Geometry: final body of the model. Coordinates: model frame, mm. Face numbers are marked on the shaded views. A direction names the side the tool comes from. Give positions to 0.01 mm unless a question says otherwise; leave off trailing zeros. Write each loop counter-clockwise with the first axis right and the second up, starting at its lowest first coordinate (ties: lowest second). Pieces come first, ordered by that corner, then holes. Notation, with made-up numbers: (66, 74) - (80, 74) arc R9 ccw to (80, 89) - close; hole circle Ø9 at (60.25, 22.5). An arc over 180 degrees is marked (long way). Return JSON: item names as keys, results as strings.
from build123d import *

# Parameters (mm, degrees)
SKETCH_1_W                = 90
SKETCH_1_H                = 40
EXTRUDE_1_DEPTH           = 51
HOLE_WIZARD_1_D           = 11
HOLE_WIZARD_1_CBORE_D     = 18
HOLE_WIZARD_1_CBORE_DEPTH = 40
HOLE_WIZARD_M10_1_D       = 8.5
HOLE_WIZARD_M10_1_DEPTH   = 24.5
HOLE_WIZARD_M10_1_TIP     = 2.553657631


with BuildPart() as part:
    # 草图1 → 凸台-拉伸1 (new body)
    with BuildSketch(Plane(origin=(0, 0, 0), x_dir=(0, 0, -1), z_dir=(1, 0, 0))):
        Rectangle(SKETCH_1_W, SKETCH_1_H)
    extrude(amount=EXTRUDE_1_DEPTH)

    # 打孔尺寸(%根据)内六角圆柱头螺钉的类型1 (through all)
    with Locations(Plane(origin=(51, 0, 0), x_dir=(0, 0, -1), z_dir=(1, 0, 0))):
        with Locations((-20, 10), (20, 10), (-20, -10), (20, -10)):
            CounterBoreHole(HOLE_WIZARD_1_D / 2, HOLE_WIZARD_1_CBORE_D / 2, HOLE_WIZARD_1_CBORE_DEPTH)

    # M10 螺纹孔1
    with Locations(Plane(origin=(51, 0, 0), x_dir=(0, 0, -1), z_dir=(1, 0, 0))):
        with Locations((-35, 0), (35, 0)):
            Hole(HOLE_WIZARD_M10_1_D / 2, depth=HOLE_WIZARD_M10_1_DEPTH)
            with Locations((0, 0, -(HOLE_WIZARD_M10_1_DEPTH + HOLE_WIZARD_M10_1_TIP / 2))):  # 118° drill point
                Cone(0, HOLE_WIZARD_M10_1_D / 2, HOLE_WIZARD_M10_1_TIP, mode=Mode.SUBTRACT)


solid = part.part
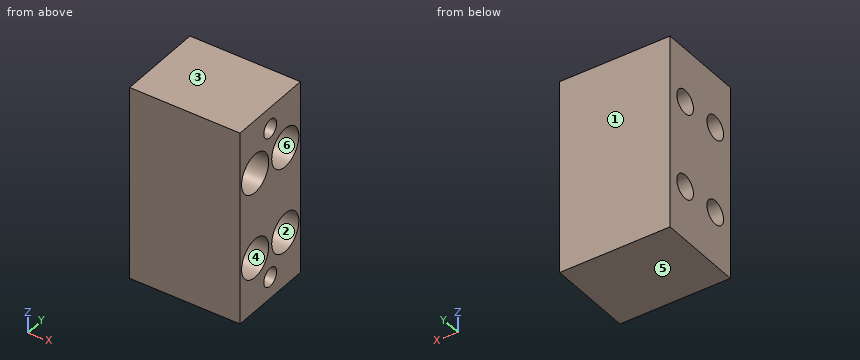
Q1. Section query D-D, the plane x = 8. Return the cut outline in (y, z), plus the area to 3 significant figures.
Answer key:
{"outline": "(-20, -45) - (20, -45) - (20, 45) - (-20, 45) - close; hole circle Ø11 at (-10, -20); hole circle Ø11 at (-10, 20); hole circle Ø11 at (10, -20); hole circle Ø11 at (10, 20)", "area": "3,220 mm^2"}
Q2. Pin query (flat end, axial travel): P1, Ø20.5, axis at y = 10, z = 20, coming from the +X side; P2, Ø5.5, axis at y = 7.5, z = 22.5, coming from the +X side; P3, Ø5, axis at y = 0, z = 35, coming from the +X side; P4, Ø10, axis at y = 10, z = 20, coming from the -X side. Return the tip coordinate at first contact, or that it passes through.
Answer key:
{"P1": "stops at x = 51", "P2": "stops at x = 11", "P3": "stops at x = 25.45", "P4": "passes through"}
Q3. Section query A-A, the plane y = 10. Return the cut outline in (x, z).
Answer key:
{"outline": "(0, -45) - (51, -45) - (51, -29) - (11, -29) - (11, -25.5) - (0, -25.5) - close; (0, -14.5) - (11, -14.5) - (11, -11) - (51, -11) - (51, 11) - (11, 11) - (11, 14.5) - (0, 14.5) - close; (0, 25.5) - (11, 25.5) - (11, 29) - (51, 29) - (51, 45) - (0, 45) - close"}
Q4. Section query B-B, the plane z = -20. Return the cut outline in (x, y), plus the area to 3 significant figures.
Answer key:
{"outline": "(0, -20) - (51, -20) - (51, -19) - (11, -19) - (11, -15.5) - (0, -15.5) - close; (0, -4.5) - (11, -4.5) - (11, -1) - (51, -1) - (51, 1) - (11, 1) - (11, 4.5) - (0, 4.5) - close; (0, 15.5) - (11, 15.5) - (11, 19) - (51, 19) - (51, 20) - (0, 20) - close", "area": "358 mm^2"}
Q5. Set-up query: the marked faces 5 and 6. Return all of +Z, -Z, +X, -X, +Y, -Y with unobstructed straight access to the full face (end or side cutting, diameter ignored); none if empty.
Answer key:
{"face 5": "-Z, +X, -X, +Y, -Y", "face 6": "+X"}
Q6. Section query C-C, the plane x = 29. Return the cut outline in (y, z).
Answer key:
{"outline": "(-20, -45) - (20, -45) - (20, 45) - (-20, 45) - close; hole circle Ø18 at (-10, -20); hole circle Ø18 at (-10, 20); hole circle Ø8.5 at (0, -35); hole circle Ø8.5 at (0, 35); hole circle Ø18 at (10, -20); hole circle Ø18 at (10, 20)"}
Q7. Material intervals for probe 1 along Z at (x, y) = (34, 0); probe 2 along Z at (x, y) = (18, -2.5); probe 3 along Y at (x, z) = (7.5, -20), sorted ascending. Write a range as [from, to].
Answer key:
{"probe 1": "z = [-45, -39.25], [-30.75, 30.75], [39.25, 45]", "probe 2": "z = [-45, -24.97], [-15.03, 15.03], [24.97, 45]", "probe 3": "y = [-20, -15.5], [-4.5, 4.5], [15.5, 20]"}
Q8. Mould query, pull axis Z, two halves, no side actions, for the marked faces 1, 2, 3 and 4. Classes: pulls with the +Z half, pulls with the -Z half, needs draft (parallel to the pull), parting line crosses it, or undercut.
Answer key:
{"face 1": "needs draft", "face 2": "undercut", "face 3": "pulls with the +Z half", "face 4": "undercut"}
